Can you work these out from the model? Positions are in its coordinate system, mm. A direction names the side the tool comes from. Round coordinates to 2 decimals unless told otherwise and drop trailing zeros. Write each loop counter-clockwise with the first axis right and the second up, starting at its lowest first coordinate (ties: lowest second). Pieces come first, ordered by that corner, then holes. Notation, with made-up numbers: (45, 87) - (95, 87) arc R27 cw to (95, 103) - close; hole circle Ø4 at (76.5, -35). An arc over 180 degrees is marked (long way). One line per item, written item: value. Start each with the question number.
(1) I want a section at A-A on z = 154.5. List the corners of the cut face in (x, y) for me.
(2) If I drill on L1, parallel to Y at x = 0, z = 149; L2, parallel to Z at x = 28, y = -7.5; L3, parallel to X at y = 1, z = 41.5, over which ranges is the centre line in solid material (lowest first)? Write a range as from..to.
(3) I want a section at B-B on z = 90. List the corners of the cut face in (x, y) for me, plus the area to 3 significant figures.
(4) Thinking about a two-plate mould opening in Y: for faces 4 (the face through (-42.33, -13.33, 0.38)), 5 (the face through (1.08, -4.88, 153.59)), 6 (the face through (5.2, 0.2, 183.5)), which applies, +Y half, -Y half, draft (parallel to the pull), parting line (faces both ways), or undercut?
(5) I'm going to push flat-ended pins straight in: pin 1 Ø4 at (y, z) = (-35.5, 154.5) entering from -X; pin 2 Ø10 at (x, z) = (-30, 111.5) entering from -Y; pin 3 Ø8 at (x, y) = (10, -38) entering from +Z. Where does each tip first touch, or does it pass through?
(6) On a 3-axis mill with a long thin cutter (end or side, diameter ignored), from which of +Z, -Z, +X, -X, +Y, -Y can I reach the whole of each face in a straight line? I mean faces 1 (the face through (-9, 9, 167)), 2 (the face through (-9, 9, 0)), 3 (the face through (-47.69, -15.02, 82.42)). Say none if no direction works.
from build123d import *

# Parameters (mm, degrees)
BODY_PROFILE_100_R              = 50
MAIN_BODY_100X167_DEPTH         = 167
SPIGOT_1_PROFILE_25_R           = 12.5
END_SPIGOT_1_25X16_5_DEPTH      = 16.5
END_START                       = 16.5
SPIGOT_2_PROFILE_25_R           = 12.5
END_SPIGOT_2_25X16_5_DEPTH      = 16.5
SPIGOT_2_DOWEL_HOLE_10X59_D     = 10
SPIGOT_2_DOWEL_HOLE_10X59_DEPTH = 59
SPIGOT_2_DOWEL_HOLE_10X59_TIP   = 3.004303095
SPIGOT_1_DOWEL_HOLE_10X59_D     = 10
SPIGOT_1_DOWEL_HOLE_10X59_DEPTH = 59
SPIGOT_1_DOWEL_HOLE_10X59_TIP   = 3.004303095
SPIGOT_EDGE_CHAMFER_0_5_SIZE    = 0.5
BODY_EDGE_CHAMFER_6_SIZE        = 6


with BuildPart() as part:
    # Body Profile Ø100 → Main Body Ø100x167 (new body)
    with BuildSketch(Plane.XY):
        with Locations(Location((0, 0, 0), (0, 0, 180))):
            Circle(BODY_PROFILE_100_R)
    extrude(amount=MAIN_BODY_100X167_DEPTH)

    # Spigot 1 Profile Ø25 → End Spigot 1 Ø25x16.5 (add)
    with BuildSketch(Plane.XY.offset(167)):
        Circle(SPIGOT_1_PROFILE_25_R)
    extrude(amount=END_SPIGOT_1_25X16_5_DEPTH)

    # Spigot 2 Profile Ø25 → End Spigot 2 Ø25x16.5 (add)
    with BuildSketch(Plane(origin=(0, 0, 0), x_dir=(-1, 0, 0), z_dir=(0, 0, -1)).offset(END_START)):
        with Locations(Location((0, 0, 0), (0, 0, 180))):
            Circle(SPIGOT_2_PROFILE_25_R)
    extrude(amount=-END_SPIGOT_2_25X16_5_DEPTH)

    # Spigot 2 Dowel Hole Ø10x59
    with Locations(Plane(origin=(0, 0, -16.5), x_dir=(-1, 0, 0), z_dir=(0, 0, -1))):
        with Locations((0, 0)):
            Hole(SPIGOT_2_DOWEL_HOLE_10X59_D / 2, depth=SPIGOT_2_DOWEL_HOLE_10X59_DEPTH)
            with Locations((0, 0, -(SPIGOT_2_DOWEL_HOLE_10X59_DEPTH + SPIGOT_2_DOWEL_HOLE_10X59_TIP / 2))):  # 118° drill point
                Cone(0, SPIGOT_2_DOWEL_HOLE_10X59_D / 2, SPIGOT_2_DOWEL_HOLE_10X59_TIP, mode=Mode.SUBTRACT)

    # Spigot 1 Dowel Hole Ø10x59
    with Locations(Plane.XY.offset(183.5)):
        with Locations((0, 0)):
            Hole(SPIGOT_1_DOWEL_HOLE_10X59_D / 2, depth=SPIGOT_1_DOWEL_HOLE_10X59_DEPTH)
            with Locations((0, 0, -(SPIGOT_1_DOWEL_HOLE_10X59_DEPTH + SPIGOT_1_DOWEL_HOLE_10X59_TIP / 2))):  # 118° drill point
                Cone(0, SPIGOT_1_DOWEL_HOLE_10X59_D / 2, SPIGOT_1_DOWEL_HOLE_10X59_TIP, mode=Mode.SUBTRACT)

    # Spigot Edge Chamfer 0.5
    spigot_edge_chamfer_0_5_edges = [part.edges().sort_by_distance(p)[0] for p in [
        (-12.5, 0, -16.5),
        (-12.5, 0, 183.5),
    ]]
    chamfer(spigot_edge_chamfer_0_5_edges, length=SPIGOT_EDGE_CHAMFER_0_5_SIZE)

    # Body Edge Chamfer 6
    body_edge_chamfer_6_edges = [part.edges().sort_by_distance(p)[0] for p in [
        (50, 0, 0),
        (50, 0, 167),
    ]]
    chamfer(body_edge_chamfer_6_edges, length=BODY_EDGE_CHAMFER_6_SIZE)


solid = part.part
Established:
1. outline: circle Ø100 at (0, 0); hole circle Ø10 at (0, 0)
2. L1: -50..-5, 5..50
2. L2: 0..167
2. L3: -49.99..-4.9, 4.9..49.99
3. outline: circle Ø100 at (0, 0)
3. area: 7,850 mm2
4. face 4: parting line
4. face 5: undercut
4. face 6: draft
5. pin 1: x = -37.12
5. pin 2: y = -43.3
5. pin 3: z = 167
6. face 1: +Z
6. face 2: -Z
6. face 3: +Z, -Z
